Geometry: final body of the model. Coordinates: model frame, mm. Face numbers are marked on the shaded views. A direction names the side the tool comes from. Give positions to 0.01 mm unless a question says otherwise; leave off trailing zeros. Write each loop counter-clockwise with the first axis right and the second up, starting at its lowest first coordinate (ties: lowest second). Pieces come first, ordered by that corner, then holes. Notation, with made-up numbers: (-16, -34.5) -> (25, -34.5) arc R32 ccw to (25, 2.5) -> close; hole circle Ø7 at (-31, 70). An arc over 180 degrees is marked (long way). Answer in a Markdown table with one row per item. Add a question column.
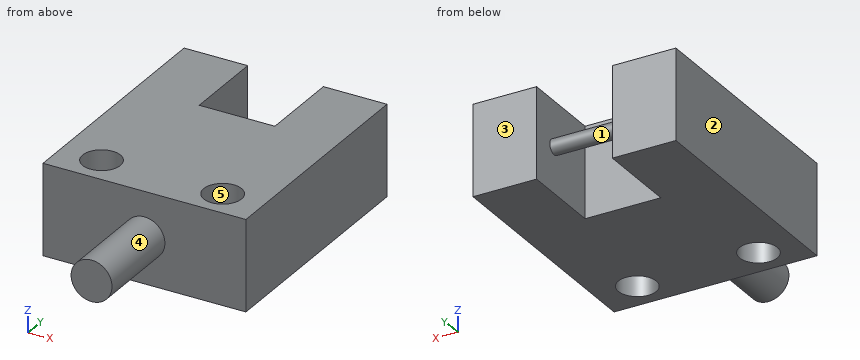
from build123d import *

# Parameters (mm, degrees)
SKETCH1_W                  = 13.4
SKETCH1_H                  = 16
BOSS_EXTRUDE1_DEPTH        = 3
SKETCH2_W                  = 5
SKETCH2_H                  = 5.5
CUT_EXTRUDE1_DEPTH         = 13.037026211
SKETCH3_R                  = 1.35
BOSS_EXTRUDE2_DEPTH        = 6
F_2_5_2_5_DIAMETER_HOLE1_D = 2.5
SKETCH6_R                  = 0.5
BOSS_EXTRUDE3_DEPTH        = 5


with BuildPart() as part:
    # Sketch1 → Boss-Extrude1 (new, symmetric)
    with BuildSketch(Plane.XY):
        Rectangle(SKETCH1_W, SKETCH1_H)
    extrude(amount=BOSS_EXTRUDE1_DEPTH, both=True)

    # Sketch2 → Cut-Extrude1 (cut, through all)
    with BuildSketch(Plane.XY.offset(3)):
        with Locations((0, 5.25)):
            Rectangle(SKETCH2_W, SKETCH2_H)
    extrude(amount=-CUT_EXTRUDE1_DEPTH, mode=Mode.SUBTRACT)

    # Sketch3 → Boss-Extrude2 (add)
    with BuildSketch(Plane.XZ.offset(8)):
        with Locations(Location((0, 0, 0), (0, 0, 90))):
            Circle(SKETCH3_R)
    extrude(amount=BOSS_EXTRUDE2_DEPTH)

    # Ø2.5 (2.5) Diameter Hole1 (through all)
    with Locations(Plane.XY.offset(3)):
        with Locations((-4, -6), (4, -6)):
            Hole(F_2_5_2_5_DIAMETER_HOLE1_D / 2)

    # Sketch6 → Boss-Extrude3 (add)
    with BuildSketch(Plane.ZY.offset(-2.5)):
        with Locations(Location((0, 6, 0), (0, 0, 90))):
            Circle(SKETCH6_R)
    extrude(amount=BOSS_EXTRUDE3_DEPTH)


solid = part.part
Q1. Contact query for a flat-ended pin moving along its axis: pin 1 Ø1.5 at (x, y) = (1, 5) entering from -Z. Output: stop coordinate, or through.
Q2. Section C-C on z = 0. Return loops of the section in (x, y), and give its area (3 significant figures).
Q3. Line query: probe 1 along X at (y, z) = (7.25, 0); probe 2 along Y at (x, z) = (-4, -1.25); probe 3 along X at (y, z) = (-7, -1.25). Output: solid intervals per line, ascending. Write a range as from..to.
Q4. Access query for the marked faces 1 and 2. Directions: +Z, -Z, +X, -X, +Y, -Y. A direction counts if a zero-diameter tool reaches every point of the face in a straight line with its end or side. Return the directions, or none.
Q5. Section D-D on y = 6.75. Return loops of the section in (x, z), and give its area (3 significant figures).
Q6. Section A-A on y = -5. Return loops of the section in (x, z).
Q7. Pull-direction query (Y, two-part tool) for the marked faces 3, 4 and 5; classes: +Y half, -Y half, draft (parallel to the pull), parting line (faces both ways), or undercut.
Q8. Section B-B on x = 0. Return loops of the section in (y, z).
Checks:
| question | item | result |
|---|---|---|
| 1 | pin 1 | z = -0.43 |
| 2 | outline | (-6.7, -8) -> (-1.35, -8) -> (-1.35, -14) -> (1.35, -14) -> (1.35, -8) -> (6.7, -8) -> (6.7, 8) -> (2.5, 8) -> (2.5, 6.5) -> (-2.5, 6.5) -> (-2.5, 8) -> (-6.7, 8) -> close; hole circle Ø2.5 at (-4, -6); hole (-2.5, 2.5) -> (2.5, 2.5) -> (2.5, 5.5) -> (-2.5, 5.5) -> close; hole circle Ø2.5 at (4, -6) |
| 2 | area | 198 mm^2 |
| 3 | probe 1 | -6.7..-2.5, 2.5..6.7 |
| 3 | probe 2 | -8..-7.25, -4.75..8 |
| 3 | probe 3 | -6.7..-4.75, -3.25..3.25, 4.75..6.7 |
| 4 | face 1 | none |
| 4 | face 2 | +Z, -Z, -X, +Y, -Y |
| 5 | outline | (-6.7, -3) -> (-2.5, -3) -> (-2.5, 3) -> (-6.7, 3) -> close; (2.5, -3) -> (6.7, -3) -> (6.7, 3) -> (2.5, 3) -> close |
| 5 | area | 50.4 mm^2 |
| 6 | outline | (-6.7, -3) -> (-4.75, -3) -> (-4.75, 3) -> (-6.7, 3) -> close; (-3.25, -3) -> (3.25, -3) -> (3.25, 3) -> (-3.25, 3) -> close; (4.75, -3) -> (6.7, -3) -> (6.7, 3) -> (4.75, 3) -> close |
| 7 | face 3 | +Y half |
| 7 | face 4 | draft |
| 7 | face 5 | undercut |
| 8 | outline | (-14, -1.35) -> (-8, -1.35) -> (-8, -3) -> (2.5, -3) -> (2.5, 3) -> (-8, 3) -> (-8, 1.35) -> (-14, 1.35) -> close; circle Ø1 at (6, 0) |
